Input: dimensioned drawing with shaded views. Units: mm. Origin: part minimum x, y, z. A direction names the side the tool comes from. Round coordinates to 2 decimals unless told otherwise and drop trailing zeros. Order: outer loops, then holes, each group sorted by start corner. A loop starts at its lowest first (then second) coordinate and runs counter-clockwise, first axis right, second up.
Item 1: Cut plane B-B on x = 4.3. Output: boundary loops of the cut face in (y, z), then the cut area to 3 significant figures.
Item 2: Line query: L1, parallel to Z at x = 4.3, y = 2; L2, parallel to Z at x = 4.3, y = 3.5; L3, parallel to Z at x = 6.5, y = 5. Output: solid intervals per line, ascending.
Item 3: Cut plane A-A on y = 4.3. Output: boundary loops of the cut face in (x, z), then the cut area to 3 significant figures.
Item 4: Cut plane D-D on z = 3. Output: boundary loops of the cut face in (x, y), then the cut area to 3 significant figures.
Item 5: Mould query, pull axis Z, two halves, no side actions, for the marked faces 3, 4 and 5. Classes: released by +Z, released by -Z, zero draft, split by the parting line, or undercut.
Item 6: Reachability of the marked faces 1 and 2 from +Z, -Z, +X, -X, +Y, -Y: full face, straight path, thin tool, end or side. Return the list, or none.
Item 7: First-contact query: pin 1 (1 mm diameter, centred on x = 7.5, z = 4, fed in from +Y); pin 2 (1 mm diameter, centred on x = 4.5, y = 6.5, fed in from +Z); pin 3 (4 mm diameter, centred on y = 7, z = 3, fed in from -X); pin 4 (2.5 mm diameter, centred on x = 4.3, z = 3, fed in from -Y). Flat tips, straight axial feed; report the tip coordinate or a pass-through.
Item 8: Cut plane C-C on z = 7.5. Output: boundary loops of the cut face in (x, y), then the cut area to 3 significant figures.
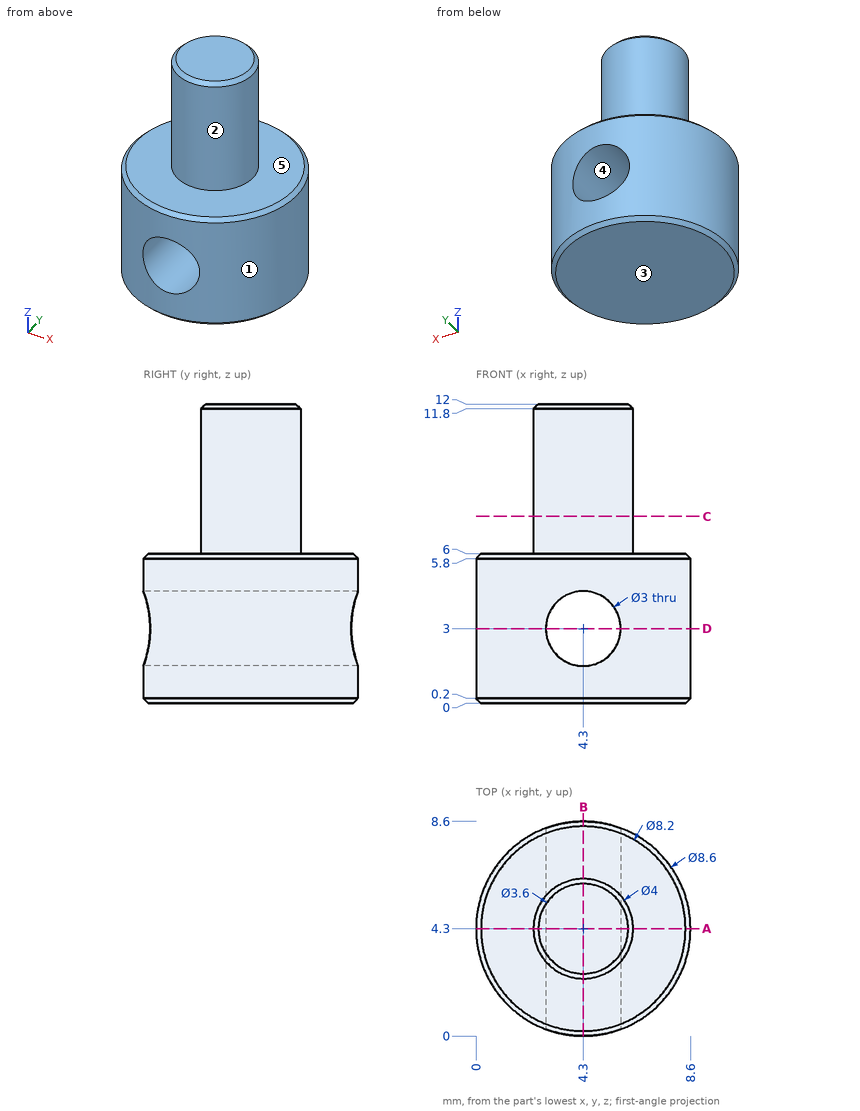
From the geometry:
1. outline: (0, 0.2) - (0.2, 0) - (8.4, 0) - (8.6, 0.2) - (8.6, 1.5) - (0, 1.5) - close; (0, 4.5) - (8.6, 4.5) - (8.6, 5.8) - (8.4, 6) - (6.3, 6) - (6.3, 11.8) - (6.1, 12) - (2.5, 12) - (2.3, 11.8) - (2.3, 6) - (0.2, 6) - (0, 5.8) - close
1. area: 49.7 mm2
2. L1: z = 0 to 1.5, 4.5 to 6
2. L2: z = 0 to 1.5, 4.5 to 12
2. L3: z = 0 to 6
3. outline: (0, 0.2) - (0.2, 0) - (8.4, 0) - (8.6, 0.2) - (8.6, 5.8) - (8.4, 6) - (6.3, 6) - (6.3, 11.8) - (6.1, 12) - (2.5, 12) - (2.3, 11.8) - (2.3, 6) - (0.2, 6) - (0, 5.8) - close; hole circle Ø3 at (4.3, 3)
3. area: 68.4 mm2
4. outline: (2.8, 0.27) - (2.8, 8.33) arc R4.3 ccw to start; (5.8, 0.27) arc R4.3 ccw to (5.8, 8.33) - close
4. area: 32.8 mm2
5. face 3: released by -Z
5. face 4: undercut
5. face 5: released by +Z
6. face 1: +Z, -Z
6. face 2: +Z
7. pin 1: stops at y = 7.65
7. pin 2: stops at z = 12
7. pin 3: stops at x = 0.06
7. pin 4: passes through
8. outline: circle Ø4 at (4.3, 4.3)
8. area: 12.6 mm2
